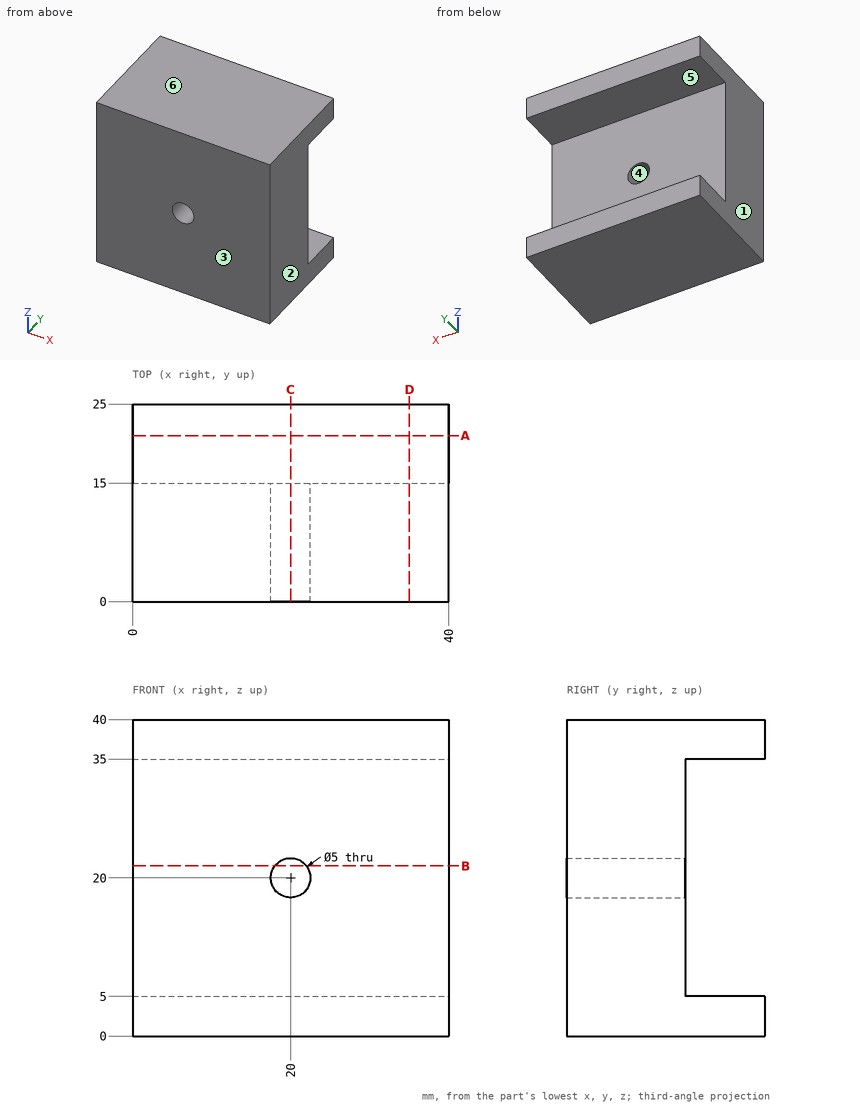
Answer from the drawing. Dimensions are ordinates in mm from the lowest x, y and z of the part. A direction names the side the tool comes from. Round coordinates to 2 decimals unless told otherwise and drop trailing zeros. Write each loop counter-clockwise with the first axis right and the second up, starting at its lowest first coordinate (ties: lowest second). Pieces come first, ordered by that corner, then holes. Notation, with made-up numbers: M 85,5 L 128,5 A34 ccw 128,35 Z; hole C 9.25,-28 d11. An arc over 180 degrees is marked long. Write each question's results on one line, items separated by ' | '. Start each with the question number.
Item 1: Given pin 1 Ø1.5 at (x, z) = (8.5, 29.5) entering from -Y; pin 2 Ø15 at (x, z) = (19, 25.5) entering from +Y, each flat-ended and moving along its own axis, determine where each tip first touches the part or whether it passes through.
Item 2: Find section B-B on z = 21.5. Write down the section's boundary in (x, y), and give its area (3 significant figures).
Item 3: Find section A-A on y = 21. Write down the section's boundary in (x, z).
Item 4: Find section C-C on x = 20. Write down the section's boundary in (y, z).
Item 5: Find section D-D on x = 35. Write down the section's boundary in (y, z), and give its area (3 significant figures).
Item 6: The mould has two halves that part along X. Classify the marked faces 1, 2, 3 and 4: +X half, -X half, draft (parallel to the pull), parting line (faces both ways), or undercut.
Item 7: Straight lines are drawn through the part: probe 1 along X at (y, z) = (5.5, 20); probe 2 along Z at (x, y) = (27, 21). For each, find the intervals that lie inside material, in ascending order.
Item 8: Which of the six approach directions +Z, -Z, +X, -X, +Y, -Y give full straight-line access (tool end or side, diameter ignored) to the marked faces 5 and 6?
Answer block:
1) pin 1: stops at y = 0 | pin 2: stops at y = 15
2) outline: M 0,0 L 18,0 L 18,15 L 0,15 Z; M 22,0 L 40,0 L 40,15 L 22,15 Z | area: 540 mm²
3) outline: M 0,0 L 40,0 L 40,5 L 0,5 Z; M 0,35 L 40,35 L 40,40 L 0,40 Z
4) outline: M 0,0 L 25,0 L 25,5 L 15,5 L 15,17.5 L 0,17.5 Z; M 0,22.5 L 15,22.5 L 15,35 L 25,35 L 25,40 L 0,40 Z
5) outline: M 0,0 L 25,0 L 25,5 L 15,5 L 15,35 L 25,35 L 25,40 L 0,40 Z | area: 700 mm²
6) face 1: -X half | face 2: +X half | face 3: draft | face 4: undercut
7) probe 1: x = 0 to 17.5, 22.5 to 40 | probe 2: z = 0 to 5, 35 to 40
8) face 5: +X, -X, +Y | face 6: +Z, +X, -X, +Y, -Y
